Work out the finished part from the listing and answer in its coordinate system (mm). A direction names the side the tool comes from. Give positions to 0.01 mm unless a question says otherwise; leave off trailing zeros.
1) Given pin 1 Ø1.1 at (y, z) = (-8, -1.5) entering from +X; pin 2 Ø6 at (x, y) = (36, -0.5) entering from -Z; pin 3 Ø5 at (x, z) = (5, -6) entering from +Y, each flat-ended and moving along its own axis, determine where each tip first touches the part or whether it passes through.
2) Straight lines are drawn through the part: probe 1 along X at (y, z) = (5.75, -4.5); probe 2 along Z at (x, y) = (18, -3); probe 3 along Y at (x, z) = (19, 0.75). For each, find the intervals that lie inside material, in ascending order.
3) A tool of negligible diameter and unlimited length cuts with its end or side. For faces 1 (the face through (5.8, 4, -7.2)), 2 (the face through (5.8, 8.2, 0)), 3 (the face through (6.1, -3.06, -7.39)), 4 (the face through (5.8, 4, 7.2)), from which of +Z, -Z, +X, -X, +Y, -Y can it reach the whole face along a straight path? Write none if from no direction.
```python
from build123d import *

# Parameters (mm, degrees)
EXTRUDE_378_DEPTH      = 6.4
SKETCH_4_W             = 0.6
SKETCH_4_H             = 11.237604307
CHAMFER_2060_SIZE      = 1.2
FILLET_2105_R          = 0.4
PATTERN_LINEAR_1_COUNT = 11
PATTERN_LINEAR_1_PITCH = 1.5


with BuildPart() as part:
    # 草图1 → Extrude 378 (new body)
    with BuildSketch(Plane(origin=(0, 0, 0), x_dir=(0, 0, -1), z_dir=(1, 0, 0))):
        Polygon((8, 4.618802154), (8, -4.618802154), (0, -9.237604307), (-8, -4.618802154), (-8, 4.618802154), (0, 9.237604307), align=None)
    extrude(amount=EXTRUDE_378_DEPTH)

    # 草图2 → 凸台-旋转1 (revolve)
    with BuildSketch(Plane.XY, mode=Mode.PRIVATE) as revolve_1_sk:
        Polygon((0, 0), (41.4, 0), (41.4, 3.701), (41.4, 5), (7.791693541, 5), (0, 5), align=None)
    revolve(revolve_1_sk.sketch.rotate(Axis((0, 0, 0), (1, 0, 0)), 90), axis=Axis((0, 0, 0), (1, 0, 0)))

    # 草图3 → 切除-旋转1 (revolve, cut)
    with BuildSketch(Plane.XY):
        Polygon((0, 8), (3.601282526, 14.237604307), (3.601282526, 19.237604307), (-10, 19.237604307), (-10, 8), align=None)
    revolve(axis=Axis((0, 0, 0), (1, 0, 0)), mode=Mode.SUBTRACT)

    # 草图5 → 切除-旋转2 (revolve, cut)
    with BuildSketch(Plane.XY):
        Polygon((6.4, 8), (2.798717474, 14.237604307), (2.798717474, 19.237604307), (12.798717474, 19.237604307), (12.798717474, 8), align=None)
    revolve(axis=Axis((0, 0, 0), (1, 0, 0)), mode=Mode.SUBTRACT)

    # 草图4 → 切除-旋转3 (revolve, cut)
    with BuildSketch(Plane.XY, mode=Mode.PRIVATE) as cut_revolve_3_sk:
        with Locations((6.1, 13.618802154)):
            Rectangle(SKETCH_4_W, SKETCH_4_H)
    revolve(cut_revolve_3_sk.sketch.rotate(Axis((0, 0, 0), (1, 0, 0)), 270), axis=Axis((0, 0, 0), (1, 0, 0)), mode=Mode.SUBTRACT)

    # Chamfer 2060
    chamfer_2060_edges = [part.edges().sort_by_distance(p)[0] for p in [
        (41.4, 0, -5),
    ]]
    chamfer(chamfer_2060_edges, length=CHAMFER_2060_SIZE)

    # Fillet 2105
    fillet_2105_edges = [part.edges().sort_by_distance(p)[0] for p in [
        (6.4, 0, -5),
    ]]
    fillet(fillet_2105_edges, radius=FILLET_2105_R)

    # 草图6 → 切除-旋转4 (revolve, cut)
    with BuildSketch(Plane.XY):
        Polygon((26.4, -3.701), (25.650022, -5), (25.650022, -6.25), (27.149978, -6.25), (27.149978, -5), align=None)
    cut_revolve_4 = revolve(axis=Axis((-3.175, 0, 0), (1, 0, 0)), mode=Mode.SUBTRACT)

    # 阵列(线性)1: 切除-旋转4 ×11
    with Locations(*[(i * PATTERN_LINEAR_1_PITCH, 0, 0) for i in range(1, PATTERN_LINEAR_1_COUNT)]):
        add(cut_revolve_4, mode=Mode.SUBTRACT)


solid = part.part
```
Results:
1. pin 1: stops at x = 6.4
1. pin 2: stops at z = -5
1. pin 3: stops at y = 7.22
2. probe 1: x = 0 to 6.4
2. probe 2: z = -4 to 4
2. probe 3: y = -4.94 to 4.94
3. face 1: -Z, +X, +Y
3. face 2: +X, +Y
3. face 3: +X
3. face 4: +Z, +X, +Y
